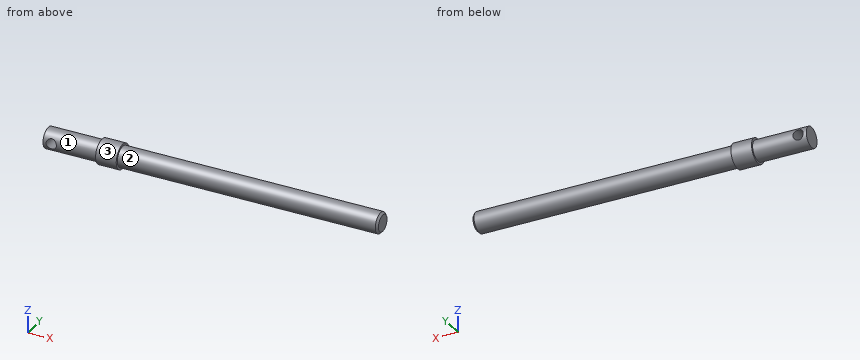
from build123d import *

# Parameters (mm, degrees)
SKETCH1_W                      = 5
SKETCH1_H                      = 3
SKETCH2_R                      = 2.5
BOSS_EXTRUDE1_DEPTH            = 13
BOSS_EXTRUDE2_START            = 63
SKETCH3_R                      = 2.5
BOSS_EXTRUDE2_DEPTH            = 63
F_2_5_2_5_DIAMETER_HOLE1_D     = 2.5
F_2_5_2_5_DIAMETER_HOLE1_DEPTH = 5.5
CHAMFER1_SIZE                  = 0.5


with BuildPart() as part:
    # Sketch1 → Revolve1 (revolve)
    with BuildSketch(Plane(origin=(0, 0, 0), x_dir=(-1, 0, 0), z_dir=(0, 0, -1)), mode=Mode.PRIVATE) as revolve1_sk:
        with Locations((-15.5, 1.5)):
            Rectangle(SKETCH1_W, SKETCH1_H)
    revolve(revolve1_sk.sketch.rotate(Axis((18, 0, 0), (-1, 0, 0)), 270), axis=Axis((18, 0, 0), (-1, 0, 0)))

    # Sketch2 → Boss-Extrude1 (add)
    with BuildSketch(Plane.ZY.offset(-13)):
        with Locations(Location((0, 0, 0), (0, 0, 180))):
            Circle(SKETCH2_R)
    extrude(amount=BOSS_EXTRUDE1_DEPTH)

    # Sketch3 → Boss-Extrude2 (add)
    with BuildSketch(Plane(origin=(18, 0, 0), x_dir=(0, 0, -1), z_dir=(1, 0, 0)).offset(BOSS_EXTRUDE2_START)):
        Circle(SKETCH3_R)
    extrude(amount=-BOSS_EXTRUDE2_DEPTH)

    # Ø2.5 (2.5) Diameter Hole1
    with Locations(Plane(origin=(2, -2.5, 0), x_dir=(-1, 0, 0), z_dir=(0, -1, 0))):
        with Locations((0, 0)):
            Hole(F_2_5_2_5_DIAMETER_HOLE1_D / 2, depth=F_2_5_2_5_DIAMETER_HOLE1_DEPTH)

    # Chamfer1
    chamfer1_edges = [part.edges().sort_by_distance(p)[0] for p in [
        (81, 0, 2.5),
    ]]
    chamfer(chamfer1_edges, length=CHAMFER1_SIZE)


solid = part.part
Check sheet for the modelled part. Datum: model origin and axes. Units: mm. Face numbers are marked on the shaded views. A direction names the side the tool comes from. Give positions to 0.01 mm unless a question says otherwise; leave off trailing zeros. Order: outer loops, then holes, each group sorted by start corner. A loop starts at its lowest first (then second) coordinate and runs counter-clockwise, first axis right, second up. Notation, with made-up numbers: (23.5, 38) - (32.5, 38) arc R19 ccw to (32.5, 61) - close; hole circle Ø2 at (88.5, -5.5). An arc over 180 degrees is marked (long way). Answer as CSV lines item,"result".
1. Go/stop test with flat-tipped pins: P1, Ø3, axis at x = 2, z = 0, coming from the -Y side; P2, Ø1, axis at x = 17.5, y = 1, coming from the +Z side; P3, Ø1, axis at x = 67.5, z = 1.5, coming from the +Y side. Record where each tip stops, or that it passes through.
Result sheet:
P1,"y = -2.5"
P2,"z = 2.96"
P3,"y = 2.29"
2. Section check A-A (z = 0). Record the boundary of the cut face in (x, y).
Result sheet:
outline,"(0, -2.5) - (0.75, -2.5) - (0.75, 2.5) - (0, 2.5) - close; (3.25, -2.5) - (13, -2.5) - (13, -3) - (18, -3) - (18, -2.5) - (80.5, -2.5) - (81, -2) - (81, 2) - (80.5, 2.5) - (18, 2.5) - (18, 3) - (13, 3) - (13, 2.5) - (3.25, 2.5) - close"
3. Section check D-D (x = 67). Record the boundary of the cut face in (y, z), then the cut area to 3 significant figures.
Result sheet:
outline,"circle Ø5 at (0, 0)"
area,"19.6 mm²"
4. Scan lines: probe 1 along Z at (x, y) = (2, 0.2); probe 2 along X at (y, z) = (-2.1, -0.5); probe 3 along Z at (x, y) = (59, 0.15). Record each from-to range of solid material in increasing order. Write a range as from..to.
Result sheet:
probe 1,"-2.49..-1.25, 1.25..2.49"
probe 2,"0..0.85, 3.15..80.84"
probe 3,"-2.5..2.5"
5. Tool access check on the marked faces 1, 2 and 3. Record the directions out of +Z, -Z, +X, -X, +Y, -Y that give a thin tool (end or side, any length) a straight path to the whole face; none if there is none.
Result sheet:
face 1,"-X"
face 2,"+X"
face 3,"+X, -X"
6. Section check B-B (y = 0). Record the boundary of the cut face in (x, z).
Result sheet:
outline,"(0, -2.5) - (13, -2.5) - (13, -3) - (18, -3) - (18, -2.5) - (80.5, -2.5) - (81, -2) - (81, 2) - (80.5, 2.5) - (18, 2.5) - (18, 3) - (13, 3) - (13, 2.5) - (0, 2.5) - close; hole circle Ø2.5 at (2, 0)"
7. Section check C-C (x = 2). Record the boundary of the cut face in (y, z), then the cut area to 3 significant figures.
Result sheet:
outline,"(-2.17, -1.25) arc R2.5 ccw to (2.17, -1.25) - close; (-2.17, 1.25) - (2.17, 1.25) arc R2.5 ccw to start"
area,"7.68 mm²"
